Geometry: final body of the model. Coordinates: model frame, mm. Coordinates: 2 decimals unless noted, no trailing zeros. Loops run counter-clockwise (first coordinate to the right, second up) from the corner with the lowest first, then second, coordinate; pieces in that order, holes last. Notation, with made-up numbers: (70, 47.25) - (107, 47.25) arc R28 cw to (107, 67.25) - close; hole circle Ø10 at (3.25, -29.5). An arc over 180 degrees is marked (long way). Answer in a Markdown table with one row per item.
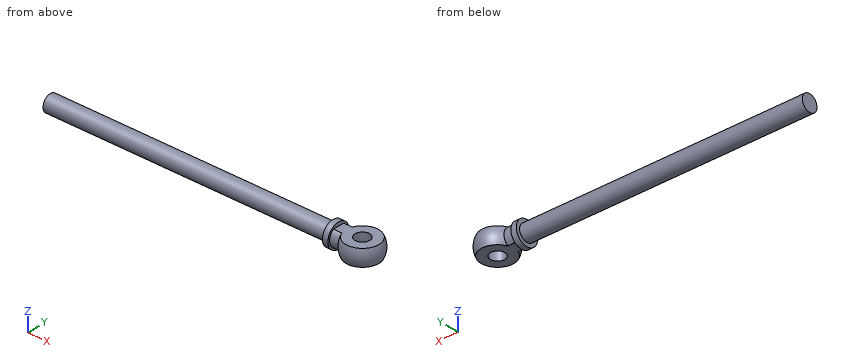
from build123d import *

# Parameters (mm, degrees)
SKETCH_2_W          = 36.907420495
SKETCH_2_H          = 136.774558304
CUT_EXTRUDE_1_DEPTH = 789.178279325
SKETCH_3_R          = 20
CUT_EXTRUDE_2_DEPTH = 754.674332852


with BuildPart() as part:
    # Sketch 1 → Revolve 1 (revolve)
    with BuildSketch(Plane.XY, mode=Mode.PRIVATE) as revolve_1_sk:
        with BuildLine():
            Line((-750, 0), (-750, 22.5))
            Line((-750, 22.5), (20, 22.5))
            Line((20, 22.5), (20, 32.5))
            Line((20, 32.5), (35, 32.5))
            Line((35, 32.5), (35, 27.5))
            Line((35, 27.5), (58.241767279, 27.5))
            ThreePointArc((58.241767279, 27.5), (114.354239164, 47.895258826), (150, 0))
            Line((150, 0), (-750, 0))
        make_face()
    revolve(revolve_1_sk.sketch.rotate(Axis((-750, 0, 0), (1, 0, 0)), 90), axis=Axis((-750, 0, 0), (1, 0, 0)))

    # Sketch 2 → Cut-Extrude 1 (cut, through all)
    with BuildSketch(Plane(origin=(35, 0, 0), x_dir=(0, 0, -1), z_dir=(1, 0, 0))):
        with Locations((40.953710247, 0)):
            Rectangle(SKETCH_2_W, SKETCH_2_H)
        with Locations((-40.953710247, 0)):
            Rectangle(SKETCH_2_W, SKETCH_2_H)
    extrude(amount=CUT_EXTRUDE_1_DEPTH, mode=Mode.SUBTRACT)

    # Sketch 3 → Cut-Extrude 2 (cut, through all)
    with BuildSketch(Plane(origin=(0, 0, -22.5), x_dir=(-1, 0, 0), z_dir=(0, 0, -1))):
        with Locations((-100, 0)):
            Circle(SKETCH_3_R)
    extrude(amount=-CUT_EXTRUDE_2_DEPTH, mode=Mode.SUBTRACT)


solid = part.part
(1) Cut plane B-B on x = 100. Output: boundary loops of the cut face in (y, z).
Verdict:
| item | result |
|---|---|
| outline | (-44.65, -22.5) - (-20, -22.5) - (-20, 22.5) - (-44.65, 22.5) arc R50 ccw to start; (20, -22.5) - (44.65, -22.5) arc R50 ccw to (44.65, 22.5) - (20, 22.5) - close |
(2) Cut plane D-D on x = -545. Output: boundary loops of the cut face in (y, z), then the cut area to 3 significant figures.
Verdict:
| item | result |
|---|---|
| outline | circle Ø45 at (0, 0) |
| area | 1,590 mm² |
(3) First-contact query: pin 1 Ø5 at (x, z) = (-311, 8) entering from +Y; pin 2 Ø1 at (y, z) = (31, 13.5) entering from +X; pin 3 Ø5 at (x, y) = (-552, 13) entering from +Z. Flat tips, straight axial feed; report the tip coordinate or a pass-through.
Verdict:
| item | result |
|---|---|
| pin 1 | stops at y = 21.82 |
| pin 2 | stops at x = 137.29 |
| pin 3 | stops at z = 19.9 |
(4) Cut plane C-C on z = 0. Output: boundary loops of the cut face in (x, y).
Verdict:
| item | result |
|---|---|
| outline | (-750, -22.5) - (20, -22.5) - (20, -32.5) - (35, -32.5) - (35, -27.5) - (58.24, -27.5) arc R50 ccw (long way) to (58.24, 27.5) - (35, 27.5) - (35, 32.5) - (20, 32.5) - (20, 22.5) - (-750, 22.5) - close; hole circle Ø40 at (100, 0) |
(5) Ray query, probe 1 along X at (y, z) = (-0.5, 4); probe 2 along Y at (x, z) = (-480.5, 10); probe 3 along Z at (x, y) = (84, -34). Return the intervals inside material, ascending.
Verdict:
| item | result |
|---|---|
| probe 1 | x = -750 to 80.01, 119.99 to 149.84 |
| probe 2 | y = -20.16 to 20.16 |
| probe 3 | z = -22.5 to 22.5 |
(6) Cut plane A-A on y = 0. Output: boundary loops of the cut face in (x, z).
Verdict:
| item | result |
|---|---|
| outline | (-750, -22.5) - (20, -22.5) - (20, -32.5) - (35, -32.5) - (35, -22.5) - (80, -22.5) - (80, 22.5) - (35, 22.5) - (35, 32.5) - (20, 32.5) - (20, 22.5) - (-750, 22.5) - close; (120, -22.5) - (144.65, -22.5) arc R50 ccw to (144.65, 22.5) - (120, 22.5) - close |
